For this review, use the dimensioned drawing (mm, ordinates from the lowest corner) and the shaded views. Coordinates: 2 decimals unless noted, no trailing zeros. Loops run counter-clockwise (first coordinate to the right, second up) from the corner with the lowest first, then second, coordinate; pieces in that order, holes last. Notation, with made-up numbers: M 48.5,74 L 73.5,74 A9 cw 73.5,79 Z; hole C 17,46 d2. An arc over 180 degrees is marked long. One line per item, written item: value.
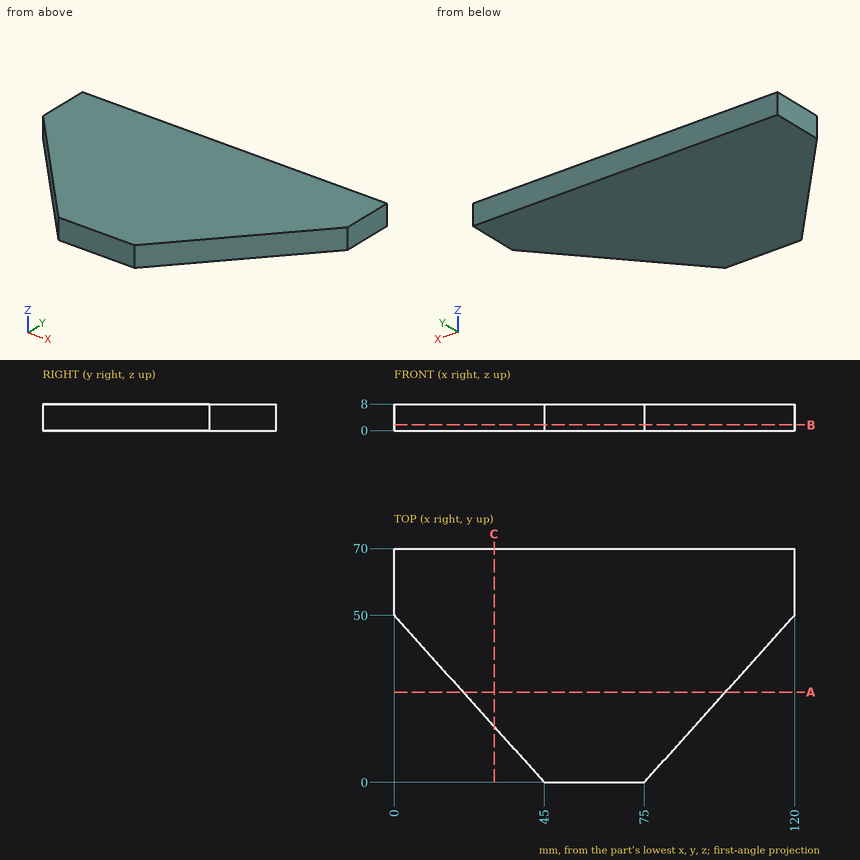
(1) We need section A-A on y = 27. State the section outline as (x, z) points, then the cut area to 3 significant figures.
Reply:
outline: M 20.7,0 L 99.3,0 L 99.3,8 L 20.7,8 Z
area: 629 mm2
(2) Insertion check: pin 1 (2 mm diameter, centred on y = 16, z = 4.5, fed in from -X); pin 2 (4 mm diameter, centred on y = 14.5, z = 5.5, fed in from -X). Each pin has a flat end and moves straight along its axis. Give the tip position at first contact, or say it passes through.
Reply:
pin 1: stops at x = 29.7
pin 2: stops at x = 30.15
(3) To check wall thickness, follow line 1 along Y through (x, z) = (93, 1.25); line 2 along X through (y, z) = (7.5, 1.5); line 3 along X through (y, z) = (24.5, 2). State the ranges of each line that lie inside material, in increasing order. Write a range as [from, to].
Reply:
line 1: y = [20, 70]
line 2: x = [38.25, 81.75]
line 3: x = [22.95, 97.05]
(4) We need section B-B on z = 1.75. State the section outline as (x, y) points, then the cut area to 3 significant figures.
Reply:
outline: M 0,50 L 45,0 L 75,0 L 120,50 L 120,70 L 0,70 Z
area: 6,150 mm2
(5) We need section C-C on x = 30. State the section outline as (y, z) points, then the cut area to 3 significant figures.
Reply:
outline: M 16.67,0 L 70,0 L 70,8 L 16.67,8 Z
area: 427 mm2
